from build123d import *

# Parameters (mm, degrees)
BASE_BLOCK_DEPTH          = 20
SIDE_BLOCK_SKETCH_W       = 40
SIDE_BLOCK_SKETCH_H       = 20
SIDE_BLOCK_DEPTH          = 20
LONG_BLOCK_SKETCH_W       = 30
LONG_BLOCK_SKETCH_H       = 30
LONG_BLOCK_DEPTH          = 35
ROUNDED_END_BOSS_DEPTH    = 20
TRIANGULAR_GUSSET_DEPTH   = 20
TRIANGULAR_CUT_12MM_DEPTH = 12


with BuildPart() as part:
    # Base Block Sketch → Base Block (new body)
    with BuildSketch(Plane.XY):
        with BuildLine():
            Line((0, 0), (105, 0))
            ThreePointArc((105, 0), (110.303300859, 2.196699141), (112.5, 7.5))
            Line((112.5, 7.5), (112.5, 32.5))
            ThreePointArc((112.5, 32.5), (110.303300859, 37.803300859), (105, 40))
            Line((105, 40), (0, 40))
            Line((0, 40), (0, 0))
        make_face()
    extrude(amount=BASE_BLOCK_DEPTH)

    # Side Block Sketch → Side Block (add)
    with BuildSketch(Plane.XZ):
        with Locations((20, 10)):
            Rectangle(SIDE_BLOCK_SKETCH_W, SIDE_BLOCK_SKETCH_H)
    extrude(amount=SIDE_BLOCK_DEPTH)

    # Long Block Sketch → Long Block (add)
    with BuildSketch(Plane.XY.offset(20)):
        with Locations((15, 25)):
            Rectangle(LONG_BLOCK_SKETCH_W, LONG_BLOCK_SKETCH_H)
    extrude(amount=LONG_BLOCK_DEPTH)

    # Rounded End Sketch → Rounded End Boss (add)
    with BuildSketch(Plane(origin=(0, 40, 0), x_dir=(1, 0, 0), z_dir=(0, 1, 0))):
        with BuildLine():
            Line((80, -20), (30, -20))
            Line((30, -20), (30, -50))
            Line((30, -50), (80, -50))
            ThreePointArc((80, -50), (87.071067812, -47.071067812), (90, -40))
            Line((90, -40), (90, -20))
            Line((90, -20), (80, -20))
        make_face()
    extrude(amount=-ROUNDED_END_BOSS_DEPTH)

    # Triangular Gusset Sketch → Triangular Gusset (add)
    with BuildSketch(Plane.ZY):
        Polygon((20, 10), (55, 10), (20, -20), align=None)
    extrude(amount=-TRIANGULAR_GUSSET_DEPTH)

    # Triangular Cut Sketch → Triangular Cut 12mm (cut)
    with BuildSketch(Plane.ZY):
        Polygon((55, 10), (20, -20), (20, 10), align=None)
    extrude(amount=-TRIANGULAR_CUT_12MM_DEPTH, mode=Mode.SUBTRACT)


solid = part.part
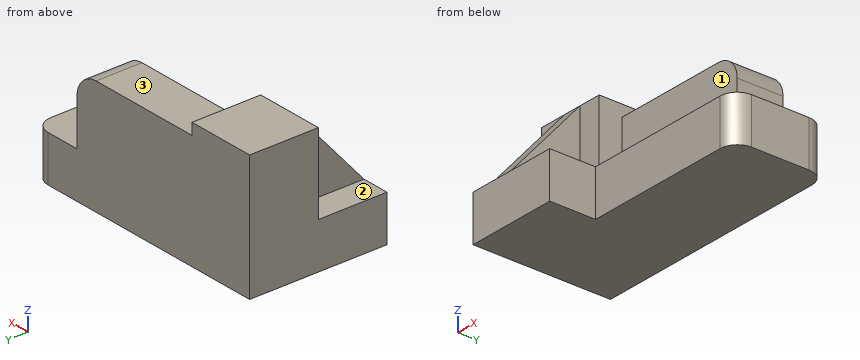
Here's how the part is built. I have some questions about the finished solid (model axes, mm). Face numbers are marked on the shaded views. A direction names the side the tool comes from. Give positions to 0.01 mm unless a question says otherwise; leave off trailing zeros. Loops run counter-clockwise (first coordinate to the right, second up) from the corner with the lowest first, then second, coordinate; pieces in that order, holes last. Notation, with made-up numbers: (32, 10) -> (77, 10) arc R24 cw to (77, 20) -> close; hole circle Ø3 at (56, 48.25). An arc over 180 degrees is marked (long way). Answer as a JSON object with one key per item and string values. Group by question number.
Item 1: I need wall thicknesses on L1, parallel to Z at x = 38, y = 13; L2, parallel to X at y = -12.5, z = 22; L3, parallel to Y at x = 90, z = 16.5. Which ranges of each line are inside material? Lowest first, please.
Item 2: Will these pins go through, and if not, where does the flat tip stop? pin 1 (15 mm diameter, centred on y = 28.5, z = 39, fed in from +X); pin 2 (12 mm diameter, centred on x = 99, y = -11.5, fed in from +Z); pin 3 (9 mm diameter, centred on y = 0.5, z = 30.5, fed in from -X); pin 4 (16 mm diameter, centred on x = 58.5, y = 26, fed in from +Z).
Item 3: Imagine slicing it at A-A on y = -5. Write out the boundary of the cut face in (x, z), then the cut area to 3 significant figures.
Item 4: On a 3-axis mill with a long thin cutter (end or side, diameter ignored), from which of +Z, -Z, +X, -X, +Y, -Y can I reach the whole of each face in a straight line? I mean the marked faces 1, 2 and 3. Say none if no direction works.
Item 5: Imagine slicing it at D-D on z = 45. Write out the boundary of the cut face in (x, y), then the cut area to 3 significant figures.
Item 6: Imagine slicing it at B-B on z = 37.5. Write out the boundary of the cut face in (x, y).
Item 7: Imagine slicing it at C-C on x = 67. Write out the boundary of the cut face in (y, z).
Answer list:
{
 "1": {"L1": "z = 0 to 20", "L2": "x = 12 to 20", "L3": "y = 0 to 40"},
 "2": {"pin 1": "stops at x = 90", "pin 2": "passes through", "pin 3": "stops at x = 12", "pin 4": "stops at z = 50"},
 "3": {"outline": "(0, 0) -> (40, 0) -> (40, 20) -> (20, 20) -> (20, 37.5) -> (12, 37.5) -> (12, 20) -> (0, 20) -> close", "area": "940 mm2"},
 "4": {"face 1": "+Z, +X, -Y", "face 2": "+Z, -X, -Y", "face 3": "+Z, +X, +Y, -Y"},
 "5": {"outline": "(0, 10) -> (12, 10) -> (12, 1.43) -> (20, 1.43) -> (20, 10) -> (30, 10) -> (30, 20) -> (88.66, 20) -> (88.66, 40) -> (0, 40) -> close", "area": "2,140 mm2"},
 "6": {"outline": "(0, 10) -> (12, 10) -> (12, -5) -> (20, -5) -> (20, 10) -> (30, 10) -> (30, 20) -> (90, 20) -> (90, 40) -> (0, 40) -> close"},
 "7": {"outline": "(0, 0) -> (40, 0) -> (40, 50) -> (20, 50) -> (20, 20) -> (0, 20) -> close"}
}
